Read the model definition and answer for the solid it produces. Units are mm, in the model's axes. A direction names the side the tool comes from. Coordinates: 2 decimals unless noted, no trailing zeros. Order: outer loops, then holes, each group sorted by start corner. A loop starts at its lowest first (then second) coordinate and runs counter-clockwise, first axis right, second up. Notation, with made-up numbers: (-16.5, 80.5) - (33.5, 80.5) arc R15 cw to (33.5, 90.5) - close; hole circle Ø2 at (-23.5, -7). An arc over 180 degrees is marked (long way). Use one line per item in the form item = value.
```python
from build123d import *

# Parameters (mm, degrees)
SKETCH_1_R      = 25
EXTRUDE_1_DEPTH = 100
SKETCH_2_R      = 7.5
EXTRUDE_2_DEPTH = 15
EXTRUDE_START   = 15
SKETCH_3_R      = 7.5
EXTRUDE_3_DEPTH = 15


with BuildPart() as part:
    # 草图1 → 凸台-拉伸1 (new body)
    with BuildSketch(Plane.XY):
        Circle(SKETCH_1_R)
    extrude(amount=EXTRUDE_1_DEPTH)

    # 草图2 → 凸台-拉伸2 (add)
    with BuildSketch(Plane.XY.offset(100)):
        Circle(SKETCH_2_R)
    extrude(amount=EXTRUDE_2_DEPTH)

    # 草图3 → 凸台-拉伸3 (add)
    with BuildSketch(Plane(origin=(0, 0, 0), x_dir=(-1, 0, 0), z_dir=(0, 0, -1)).offset(EXTRUDE_START)):
        with Locations(Location((0, 0, 0), (0, 0, 180))):
            Circle(SKETCH_3_R)
    extrude(amount=-EXTRUDE_3_DEPTH)


solid = part.part
```
(1) Which of the six approach directions +Z, -Z, +X, -X, +Y, -Y give full straight-line access (tool end or side, diameter ignored) to faces 1 (the cylindrical face through (-7.493, 0.33, 107.395)), 2 (the flat face through (-6, -5, 0)), 3 (the flat face through (0, 0, 115))?
Answer list:
face_1 = +Z
face_2 = -Z
face_3 = +Z, +X, -X, +Y, -Y
(2) Given pin 1 Ø3 at (x, z) = (11, 91) entering from -Y; pin 2 Ø1.5 at (x, y) = (17, 7.5) entering from -Z; pin 3 Ø3 at (y, z) = (7.5, 38.5) entering from -X, each flat-ended and moving along its own axis, determine where each tip first touches the part or whether it passes through.
Answer list:
pin_1 = -23.12
pin_2 = 0
pin_3 = -24.27
(3) Straight lines are drawn through the part: L1, parallel to Y at x = 0, z = 2; L2, parallel to Z at x = -5, y = -10; L3, parallel to X at y = -20, z = 56. For each, find the intervals that lie inside material, in ascending order.
Answer list:
L1 = -25 to 25
L2 = 0 to 100
L3 = -15 to 15
(4) Section D-D, the plane y = 12 is taken. Write down the section's boundary in (x, z), then the cut area to 3 significant figures.
Answer list:
outline = (-21.93, 0) - (21.93, 0) - (21.93, 100) - (-21.93, 100) - close
area = 4,390 mm2
(5) Section A-A, the plane y = 0 is taken. Write down the section's boundary in (x, z).
Answer list:
outline = (-25, 0) - (-7.5, 0) - (-7.5, -15) - (7.5, -15) - (7.5, 0) - (25, 0) - (25, 100) - (7.5, 100) - (7.5, 115) - (-7.5, 115) - (-7.5, 100) - (-25, 100) - close
(6) Section C-C, the plane z = 61 is taken. Write down the section's boundary in (x, y), then the cut area to 3 significant figures.
Answer list:
outline = circle Ø50 at (0, 0)
area = 1,960 mm2
